```python
from build123d import *

# Parameters (mm, degrees)
SKETCH1_W                                            = 15
SKETCH1_H                                            = 15.5
BOSS_EXTRUDE1_DEPTH                                  = 6
SKETCH2_W                                            = 15
SKETCH2_H                                            = 4
BOSS_EXTRUDE2_DEPTH                                  = 9
SKETCH3_R                                            = 3.25
CUT_EXTRUDE1_DEPTH                                   = 1
HOLE_SIZE_PER_SOCKET_HEAD_CAP_SCREW_TYPE_D           = 3.4
HOLE_SIZE_PER_SOCKET_HEAD_CAP_SCREW_TYPE_CBORE_D     = 6
HOLE_SIZE_PER_SOCKET_HEAD_CAP_SCREW_TYPE_CBORE_DEPTH = 3.4
CHAMFER1_SIZE                                        = 5
CHAMFER2_SIZE                                        = 1
CHAMFER3_SIZE                                        = 0.5


with BuildPart() as part:
    # Sketch1 → Boss-Extrude1 (new body)
    with BuildSketch(Plane.XY):
        Rectangle(SKETCH1_W, SKETCH1_H)
    extrude(amount=BOSS_EXTRUDE1_DEPTH)

    # Sketch2 → Boss-Extrude2 (add)
    with BuildSketch(Plane.XY.offset(6)):
        with Locations((0, -5.75)):
            Rectangle(SKETCH2_W, SKETCH2_H)
    extrude(amount=BOSS_EXTRUDE2_DEPTH)

    # Sketch3 → Cut-Extrude1 (cut)
    with BuildSketch(Plane(origin=(0, -3.75, 0), x_dir=(1, 0, 0), z_dir=(0, 1, 0))):
        with Locations(Location((0, -11, 0), (0, 0, 270))):
            Circle(SKETCH3_R)
    extrude(amount=-CUT_EXTRUDE1_DEPTH, mode=Mode.SUBTRACT)

    # Hole size per socket head cap screw type 1 (through all)
    with Locations(Plane(origin=(0, -7.75, 0), x_dir=(-1, 0, 0), z_dir=(0, -1, 0))):
        with Locations((4, -3.5), (-4, -3.5)):
            CounterBoreHole(HOLE_SIZE_PER_SOCKET_HEAD_CAP_SCREW_TYPE_D / 2, HOLE_SIZE_PER_SOCKET_HEAD_CAP_SCREW_TYPE_CBORE_D / 2, HOLE_SIZE_PER_SOCKET_HEAD_CAP_SCREW_TYPE_CBORE_DEPTH)

    # Chamfer1
    chamfer1_edges = [part.edges().sort_by_distance(p)[0] for p in [
        (-7.5, -5.75, 15),
        (7.5, -5.75, 15),
    ]]
    chamfer(chamfer1_edges, length=CHAMFER1_SIZE)

    # Chamfer2
    chamfer2_edges = [part.edges().sort_by_distance(p)[0] for p in [
        (-7.5, 0, 0),
        (7.5, 0, 0),
    ]]
    chamfer(chamfer2_edges, length=CHAMFER2_SIZE)

    # Chamfer3
    chamfer3_edges = [part.edges().sort_by_distance(p)[0] for p in [
        (0, 7.75, 6),
        (0, 7.75, 0),
    ]]
    chamfer(chamfer3_edges, length=CHAMFER3_SIZE)


solid = part.part
```
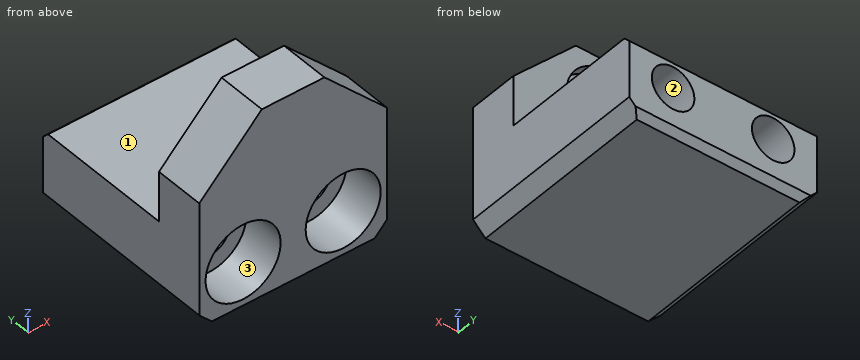
Can you work these out from the model? Positions are in its coordinate system, mm. Face numbers are marked on the shaded views. A direction names the side the tool comes from. Coordinates: 2 decimals unless noted, no trailing zeros. Loops run counter-clockwise (first coordinate to the right, second up) from the corner with the lowest first, then second, coordinate; pieces in that order, holes last. Notation, with made-up numbers: (-21, 83) -> (37, 83) arc R17 ccw to (37, 114) -> close; hole circle Ø5 at (30, -32.75). An arc over 180 degrees is marked (long way). Answer as a JSON object with one key per item and string values.
1) For P1, Ø1, axis at x = -5.5, z = 12.5, coming from the +Y side; P2, Ø3.5, axis at x = 3, y = 3.5, coming from the +Z side; P3, Ø4, axis at x = -4, z = 3.5, coming from the -Y side, each with a flat end and sliding along its axis, tell me the tip position at first contact or that it passes through.
Results:
{"P1": "stops at y = -3.75", "P2": "stops at z = 6", "P3": "stops at y = -4.35"}
2) Imagine slicing it at A-A (x = -4). Please give me the cut outline in (y, z), then the cut area to 3 significant figures.
Results:
{"outline": "(-7.75, 0) -> (7.25, 0) -> (7.75, 0.5) -> (7.75, 1.8) -> (-4.35, 1.8) -> (-4.35, 0.5) -> (-7.75, 0.5) -> close; (-7.75, 6.5) -> (-4.35, 6.5) -> (-4.35, 5.2) -> (7.75, 5.2) -> (7.75, 5.5) -> (7.25, 6) -> (-3.75, 6) -> (-3.75, 13.5) -> (-7.75, 13.5) -> close", "area": "61.2 mm^2"}
3) If I drill on line 1 (Z direction, x = -4, y = 0); line 2 (X direction, y = 5.25, z = 3.25); line 3 (X direction, y = -4.5, z = 11), over which ranges is the centre line in solid material (lowest first)?
Results:
{"line 1": "z = 0 to 1.8, 5.2 to 6", "line 2": "x = -7.5 to -5.68, -2.32 to 2.32, 5.68 to 7.5", "line 3": "x = -6.5 to -3.25, 3.25 to 6.5"}
4) Imagine slicing it at C-C (z = 3.5). Please give me the cut outline in (x, y).
Results:
{"outline": "(-7.5, -7.75) -> (-7, -7.75) -> (-7, -4.35) -> (-5.7, -4.35) -> (-5.7, 7.75) -> (-7.5, 7.75) -> close; (-2.3, -4.35) -> (-1, -4.35) -> (-1, -7.75) -> (1, -7.75) -> (1, -4.35) -> (2.3, -4.35) -> (2.3, 7.75) -> (-2.3, 7.75) -> close; (5.7, -4.35) -> (7, -4.35) -> (7, -7.75) -> (7.5, -7.75) -> (7.5, 7.75) -> (5.7, 7.75) -> close"}
5) Imagine slicing it at B-B (y = -6). Please give me the cut outline in (x, z).
Results:
{"outline": "(-7.5, 1) -> (-6.5, 0) -> (6.5, 0) -> (7.5, 1) -> (7.5, 10) -> (2.5, 15) -> (-2.5, 15) -> (-7.5, 10) -> close; hole circle Ø6 at (-4, 3.5); hole circle Ø6 at (4, 3.5)"}
6) For the marked faces 1, 2 and 3, which set-ups out of +Z, -Z, +X, -X, +Y, -Y let a thin tool reach every point of the face, with its end or its side?
Results:
{"face 1": "+Z, +X, -X, +Y", "face 2": "+Y, -Y", "face 3": "-Y"}
7) Imagine slicing it at D-D (x = 0). Please give me the cut outline in (y, z).
Results:
{"outline": "(-7.75, 0) -> (7.25, 0) -> (7.75, 0.5) -> (7.75, 5.5) -> (7.25, 6) -> (-3.75, 6) -> (-3.75, 7.75) -> (-4.75, 7.75) -> (-4.75, 14.25) -> (-3.75, 14.25) -> (-3.75, 15) -> (-7.75, 15) -> close"}
